Part model, mm, in its own coordinate system. A direction names the side the tool comes from. Round coordinates to 2 decimals unless told otherwise and drop trailing zeros. Order: outer loops, then holes, each group sorted by start corner. A loop starts at its lowest first (then second) coordinate and runs counter-clockwise, first axis right, second up. Notation, with made-up numbers: M 48,-15.5 L 92,-15.5 A15 ccw 92,9.5 Z; hole C 89.5,35.5 d5. An arc over 180 degrees is marked long. One line per question, with ' | ' between items.
from build123d import *

# Parameters (mm, degrees)
SKETCH1_W               = 11.793584223
SKETCH1_H               = 7.577709462
BOSS_EXTRUDE1_DEPTH     = 10
SHELL1_T                = -0.5
CUT_EXTRUDE1_DEPTH      = 47.145900644
CUT_EXTRUDE1_DEPTH_BACK = 47.145900644
SKETCH3_R               = 0.739402186
BOSS_EXTRUDE2_DEPTH     = 0.5
CUT_EXTRUDE2_DEPTH      = 47.256828104
CUT_EXTRUDE2_DEPTH_BACK = 47.256828104
SKETCH4_R               = 0.342163572
CUT_EXTRUDE3_DEPTH      = 18.219474717
CUT_EXTRUDE3_DEPTH_BACK = 0.5
SKETCH5_R               = 0.838133872
SKETCH6_R               = 1.176594154
BOSS_EXTRUDE3_DEPTH     = 1.5
SKETCH7_R               = 2
BOSS_EXTRUDE4_DEPTH     = 3
SKETCH8_R               = 2.5
BOSS_EXTRUDE5_DEPTH     = 3
SKETCH9_R               = 2.944420976
BOSS_EXTRUDE6_DEPTH     = 3.293584224


with BuildPart() as part:
    # Sketch1 → Boss-Extrude1 (new body)
    with BuildSketch(Plane.XY):
        with Locations((-38.510667459, -3.788854731)):
            Rectangle(SKETCH1_W, SKETCH1_H)
    extrude(amount=-BOSS_EXTRUDE1_DEPTH)

    # Shell1
    shell1_openings = [part.faces().sort_by_distance(p)[0] for p in [
        (-38.510667459, -7.577709462, -5),
    ]]
    offset(amount=SHELL1_T, openings=shell1_openings, kind=Kind.INTERSECTION)

    # Sketch2 → Cut-Extrude1 (cut, two sides: drawn at the far end of the back side and taken through both)
    with BuildSketch(Plane.XY.offset(-CUT_EXTRUDE1_DEPTH_BACK)):
        Polygon((-32.613875348, -7.577709462), (-43.28798944, -6.09867093), (-43.492929631, -7.577709462), (-42.32222074, -12.914238607), (-34.209763667, -9.465064681), align=None)
    extrude(amount=CUT_EXTRUDE1_DEPTH + CUT_EXTRUDE1_DEPTH_BACK, mode=Mode.SUBTRACT)

    # Sketch3 → Boss-Extrude2 (add)
    with BuildSketch(Plane.XY):
        with Locations(Location((-43.348851562, -4.90387791, 0), (0, 0, 180))):
            Circle(SKETCH3_R)
    extrude(amount=BOSS_EXTRUDE2_DEPTH)

    # Sketch4 → Cut-Extrude2 (cut, two sides: drawn at the far end of the back side and taken through both)
    with BuildSketch(Plane.XY.offset(0.5).offset(-CUT_EXTRUDE2_DEPTH_BACK)):
        with Locations((-43.348851562, -4.90387791)):
            Circle(SKETCH4_R)
    extrude(amount=CUT_EXTRUDE2_DEPTH + CUT_EXTRUDE2_DEPTH_BACK, mode=Mode.SUBTRACT)

    # Sketch5 → Cut-Extrude3 (cut, two sides: drawn at the far end of the back side and taken through both)
    with BuildSketch(Plane(origin=(-32.613875348, 0, 0), x_dir=(0, 0, -1), z_dir=(1, 0, 0)).offset(-CUT_EXTRUDE3_DEPTH_BACK)):
        with Locations(Location((5, -3.788854731, 0), (0, 0, 180))):
            Circle(SKETCH5_R)
    extrude(amount=CUT_EXTRUDE3_DEPTH + CUT_EXTRUDE3_DEPTH_BACK, mode=Mode.SUBTRACT)

    # Sketch6 → Boss-Extrude3 (add)
    with BuildSketch(Plane(origin=(-43.907459571, 0, 0), x_dir=(0, 0, -1), z_dir=(1, 0, 0))):
        with Locations(Location((5, -4.038854731, 0), (0, 0, 180))):
            Circle(SKETCH6_R)
    extrude(amount=BOSS_EXTRUDE3_DEPTH)

    # Sketch7 → Boss-Extrude4 (add)
    with BuildSketch(Plane(origin=(-42.407459571, 0, 0), x_dir=(0, 0, -1), z_dir=(1, 0, 0))):
        with Locations((5, -4.038854731)):
            Circle(SKETCH7_R)
    extrude(amount=BOSS_EXTRUDE4_DEPTH)

    # Sketch8 → Boss-Extrude5 (add)
    with BuildSketch(Plane(origin=(-39.407459571, 0, 0), x_dir=(0, 0, -1), z_dir=(1, 0, 0))):
        with Locations((5, -4.038854731)):
            Circle(SKETCH8_R)
    extrude(amount=BOSS_EXTRUDE5_DEPTH)

    # Sketch9 → Boss-Extrude6 (add)
    with BuildSketch(Plane(origin=(-36.407459571, 0, 0), x_dir=(0, 0, -1), z_dir=(1, 0, 0))):
        with Locations((5, -4.038854731)):
            Circle(SKETCH9_R)
    extrude(amount=BOSS_EXTRUDE6_DEPTH)


solid = part.part
1) Which spindle directions (+Z, -Z, +X, -X, +Y, -Y) get a long thin tool onto all of the face, cutting with end or side? Do faces 4 (the face through (-44.03, -4.62, 0.25)), 5 (the face through (-39, -4, -9.5)), 6 (the face through (-41, -4, -3)), 7 (the face through (-32.787, -7.554, -5.023)), 8 (the face through (-32.614, -5, -5)). Say none if no direction does.
The answers:
face 4: +Z | face 5: -Y | face 6: none | face 7: +Z, -Z, -Y | face 8: +Z, -Z, +X, +Y, -Y
2) Two-plate mould, pull along Y, no slides. Class faces 1 (the face through (-44.2, -7.578, -4.9)), 2 (the face through (-39, -4, 0)), 3 (the face through (-32.87, -4.04, -4.2)): released by +Y, released by -Y, zero draft, split by the parting line, or undercut.
The answers:
face 1: released by -Y | face 2: zero draft | face 3: undercut
3) Drop flat-ended pins along their axis: pin 1 (1.3 mm diameter, centred on y = -3.79, z = -5, fed in from +X); pin 2 (2 mm diameter, centred on x = -40.5, y = -5.5, fed in from +Z). Give the stop position or say it passes through.
The answers:
pin 1: stops at x = -33.11 | pin 2: stops at z = 0
4) Saw through at A-A (z = -5). List the corners of the cut face in (x, y).
The answers:
outline: M -44.41,-7.58 L -43.91,-7.58 L -43.91,-5.22 L -42.41,-5.22 L -42.41,-6.04 L -39.41,-6.04 L -39.41,-6.54 L -36.41,-6.54 L -36.41,-6.98 L -33.11,-6.98 L -33.11,-7.51 L -32.61,-7.58 L -32.61,-4.63 L -33.11,-4.63 L -33.11,-2.95 L -32.61,-2.95 L -32.61,0 L -44.41,0 Z; hole M -43.91,-2.86 L -42.41,-2.86 L -42.41,-2.04 L -39.41,-2.04 L -39.41,-1.54 L -36.41,-1.54 L -36.41,-1.09 L -33.11,-1.09 L -33.11,-0.5 L -43.91,-0.5 Z
5) Saw through at B-B (x = -38). List the corners of the cut face in (y, z).
The answers:
outline: M -6.83,-10 L 0,-10 L 0,0 L -6.83,0 L -6.83,-0.5 L -0.5,-0.5 L -0.5,-9.5 L -6.83,-9.5 Z; C -4.04,-5 d5
6) Saw through at D-D (x = -34.25). List the corners of the cut face in (y, z).
The answers:
outline: M -7.35,-10 L 0,-10 L 0,0 L -7.35,0 L -7.35,-0.5 L -0.5,-0.5 L -0.5,-9.5 L -7.35,-9.5 Z; C -4.04,-5 d5.89
7) Saw through at C-C (z = -1). List the corners of the cut face in (x, y).
The answers:
outline: M -44.41,-7.58 L -43.91,-7.58 L -43.91,-0.5 L -33.11,-0.5 L -33.11,-7.51 L -32.61,-7.58 L -32.61,0 L -44.41,0 Z
8) Probe line 1 (X direction, y = -0.75, z = -4); line 2 (X direction, y = -5.5, z = -5.75); line 3 (Z direction, x = -34.75, y = -5.5). List the from-to ranges inside material, lowest first. Write a range as [from, to].
The answers:
line 1: x = [-44.41, -43.91], [-33.11, -32.61] | line 2: x = [-44.41, -43.91], [-42.41, -32.61] | line 3: z = [-10, -9.5], [-7.56, -2.44], [-0.5, 0]
